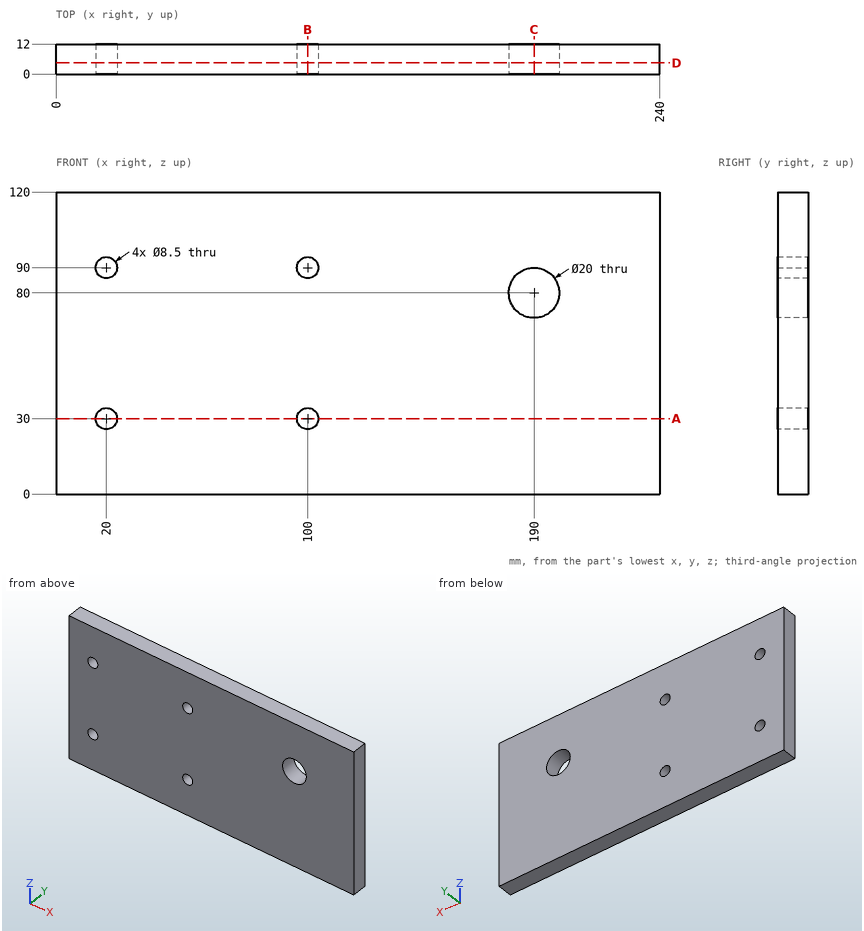
Here's the drawing with two shaded views (mm, measured from the low corner). I have some questions. Coordinates: 2 decimals unless noted, no trailing zeros. Loops run counter-clockwise (first coordinate to the right, second up) from the corner with the lowest first, then second, coordinate; pieces in that order, holes last.
Item 1: Suppose I cut it at D-D (y = 4.5). Please give me the cut outline in (x, z).
Answers below:
outline: (0, 0) - (240, 0) - (240, 120) - (0, 120) - close; hole circle Ø8.5 at (20, 30); hole circle Ø8.5 at (20, 90); hole circle Ø8.5 at (100, 30); hole circle Ø8.5 at (100, 90); hole circle Ø20 at (190, 80)
Item 2: I'm going to push a flat-ended pin straight in: pin 1 (7 mm diameter, centred on x = 100, z = 30, fed in from +Y). Where does the tip first touch, or does it pass through?
Answers below:
pin 1: passes through
Item 3: Suppose I cut it at C-C (x = 190). Please give me the cut outline in (y, z).
Answers below:
outline: (0, 0) - (12, 0) - (12, 70) - (0, 70) - close; (0, 90) - (12, 90) - (12, 120) - (0, 120) - close
Item 4: Suppose I cut it at A-A (z = 30). Please give me the cut outline in (x, y), then the cut area to 3 significant figures.
Answers below:
outline: (0, 0) - (15.75, 0) - (15.75, 12) - (0, 12) - close; (24.25, 0) - (95.75, 0) - (95.75, 12) - (24.25, 12) - close; (104.25, 0) - (240, 0) - (240, 12) - (104.25, 12) - close
area: 2,680 mm2
Item 5: Suppose I cut it at B-B (x = 100). Please give me the cut outline in (y, z), then the cut area to 3 significant figures.
Answers below:
outline: (0, 0) - (12, 0) - (12, 25.75) - (0, 25.75) - close; (0, 34.25) - (12, 34.25) - (12, 85.75) - (0, 85.75) - close; (0, 94.25) - (12, 94.25) - (12, 120) - (0, 120) - close
area: 1,240 mm2
Item 6: Please list where these lines run through material, in increasing order: L1, parallel to X at y = 6, z = 30; L2, parallel to X at y = 6.25, z = 33.5; L3, parallel to X at y = 4.5, z = 80.
Answers below:
L1: x = 0 to 15.75, 24.25 to 95.75, 104.25 to 240
L2: x = 0 to 17.59, 22.41 to 97.59, 102.41 to 240
L3: x = 0 to 180, 200 to 240
